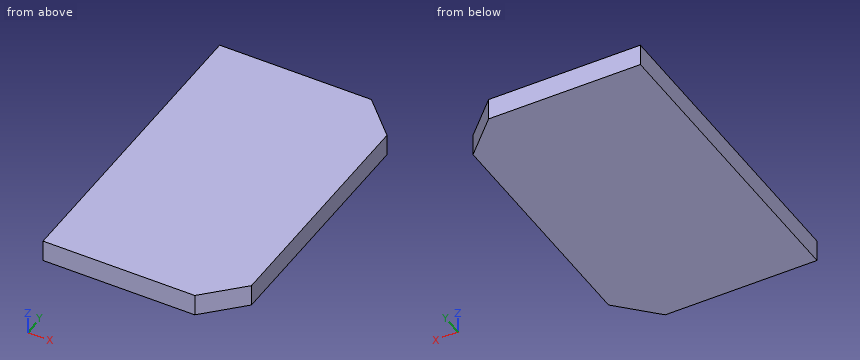
```python
from build123d import *

# Parameters (mm, degrees)
SKETCH_1_W      = 26
SKETCH_1_H      = 43
EXTRUDE_1_DEPTH = 3
CHAMFER_1_SIZE  = 5


with BuildPart() as part:
    # 草图1 → 凸台-拉伸1 (new body)
    with BuildSketch(Plane.XY):
        with Locations((13, 21.5)):
            Rectangle(SKETCH_1_W, SKETCH_1_H)
    extrude(amount=EXTRUDE_1_DEPTH)

    # 倒角1
    chamfer_1_edges = [part.edges().sort_by_distance(p)[0] for p in [
        (26, 43, 1.5),
        (26, 0, 1.5),
    ]]
    chamfer(chamfer_1_edges, length=CHAMFER_1_SIZE)


solid = part.part
```
Check sheet for the modelled part. Datum: model origin and axes. Units: mm. Round coordinates to 2 decimals unless told otherwise and drop trailing zeros. Write each loop counter-clockwise with the first axis right and the second up, starting at its lowest first coordinate (ties: lowest second). Pieces come first, ordered by that corner, then holes. Notation, with made-up numbers: M -24.5,42 L 9.5,42 A8 ccw 9.5,51 Z; hole C 73.25,-2.5 d7. An arc over 180 degrees is marked long. Write item = value, one per line. Start each with the question number.
1. Section check A-A, the plane x = 22.75. Record the cut outline in (y, z).
2. Section check B-B, the plane z = 0.55. Record the cut outline in (x, y).
3. Scan lines: line 1 (X direction, y = 2.5, z = 0.25); line 2 (X direction, y = 4, z = 0.3); line 3 (Y direction, x = 22, z = 2.7). Record each from-to range of solid material in increasing order. Write a range as [from, to].
Results found:
q1.outline = M 1.75,0 L 41.25,0 L 41.25,3 L 1.75,3 Z
q2.outline = M 0,0 L 21,0 L 26,5 L 26,38 L 21,43 L 0,43 Z
q3.line_1 = [0, 23.5]
q3.line_2 = [0, 25]
q3.line_3 = [1, 42]
